The drawing under review shows one solid part. Ordinate dimensions are in mm from its lowest x, y, z. Give positions to 0.01 mm unless a question says otherwise; leave off trailing zeros. Loops run counter-clockwise (first coordinate to the right, second up) from the corner with the lowest first, then second, coordinate; pieces in that order, holes last. Notation, with made-up numbers: M 25.5,-37 L 50.5,-37 A7 cw 50.5,-29 Z; hole C 82.25,55 d6. An arc over 180 degrees is marked long. Write item = value, one per line. Start each with the question number.
1. We need section A-A on z = 114. Give the boundary of the cut face in (x, y), then the cut area to 3 significant figures.
2. We need section C-C on z = 15. Give the boundary of the cut face in (x, y), then the cut area to 3 significant figures.
3. We need section D-D on y = 49. Give the boundary of the cut face in (x, z).
4. For pin 1 (3 mm diameter, centred on x = 94.5, z = 104, fed in from +Y); pin 2 (1.5 mm diameter, centred on x = 39.5, y = 19.5, fed in from -Z); pin 3 (11 mm diameter, centred on x = 62, z = 15, fed in from -Y); pin 4 (3 mm diameter, centred on x = 91.5, z = 27, fed in from +Y), all flat-tipped, find the tip position at first contact; note any pin that passes through.
5. Draft analysis for pull direction X (two halves, no side actions). For the marked faces 1, 2, 3 and 4, state which applies: pulls with the +X half, pulls with the -X half, needs draft (parallel to the pull), parting line crosses it, or undercut.
6. Wall thickness on line 1 along X through (y, z) = (3, 114); line 2 along X through (y, z) = (31, 47); line 3 along X through (y, z) = (3, 15): over which ranges is each line inside the solid? List them lowest first. Write a range as from..to.
7. We need section B-B on x = 109. Give the boundary of the cut face in (y, z), then the cut area to 3 significant figures.
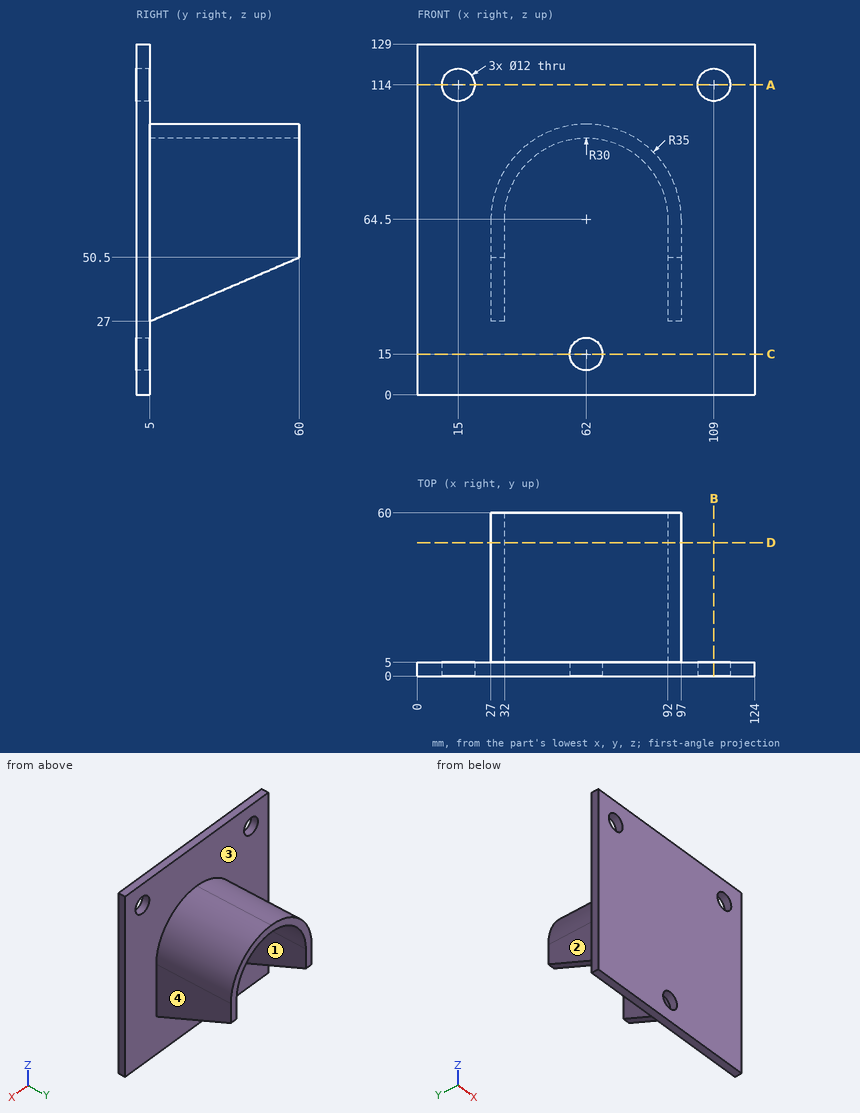
Final values:
q1.outline = M 0,0 L 9,0 L 9,5 L 0,5 Z; M 21,0 L 103,0 L 103,5 L 21,5 Z; M 115,0 L 124,0 L 124,5 L 115,5 Z
q1.area = 500 mm²
q2.outline = M 0,0 L 56,0 L 56,5 L 0,5 Z; M 68,0 L 124,0 L 124,5 L 68,5 Z
q2.area = 560 mm²
q3.outline = M 27,45.8 L 32,45.8 L 32,64.5 A30 cw 92,64.5 L 92,45.8 L 97,45.8 L 97,64.5 A35 ccw 27,64.5 Z
q4.pin_1 = 5
q4.pin_2 = 83.46
q4.pin_3 = through
q4.pin_4 = 8.31
q5.face_1 = undercut
q5.face_2 = pulls with the -X half
q5.face_3 = undercut
q5.face_4 = pulls with the +X half
q6.line_1 = 0..9, 21..103, 115..124
q6.line_2 = 27..32, 92..97
q6.line_3 = 0..56, 68..124
q7.outline = M 0,0 L 5,0 L 5,108 L 0,108 Z; M 0,120 L 5,120 L 5,129 L 0,129 Z
q7.area = 585 mm²
